Here's how the part is built. I have some questions about the finished solid (model axes, mm). A direction names the side the tool comes from. Round coordinates to 2 decimals unless told otherwise and drop trailing zeros. Loops run counter-clockwise (first coordinate to the right, second up) from the corner with the lowest first, then second, coordinate; pieces in that order, holes last. Notation, with made-up numbers: (62.25, 81) - (71.25, 81) arc R15 ccw to (71.25, 90) - close; hole circle Ø2 at (23.5, -9.75). An arc over 180 degrees is marked (long way). Answer as a JSON object with one key per item and string values. Group by question number.
1) I want a section at A-A, the plane z = 0. Please give me the cut outline in (x, y).
2) Will this pin go through, and if not, where does the flat tip stop? P1, Ø3, axis at x = 7, z = -2.5, coming from the -Y side.
3) If I drill on line 1 along X through (y, z) = (-3.75, -5.5); line 2 along Y through (x, z) = (13.5, 0.25); line 3 along Z through (x, y) = (1, 0.25), over which ranges is the centre line in solid material (lowest first)? Write a range as [from, to].
4) If we mould it in two halves opening along X, with no side actions, what happens to faces 1 (the face through (0, 0, 0)), 2 (the face through (24.74, 6.21, 3.23)), 3 (the face through (21.058, 3.955, -5.158)), 4 (the face through (28, 0, 0))? For each: pulls with the +X half, pulls with the -X half, needs draft (parallel to the pull), parting line crosses it, or undercut.
5) I want a section at C-C, the plane x = 14. Please give me the cut outline in (y, z).
6) Which directions (+Z, -Z, +X, -X, +Y, -Y) give clear straight access to the entire face, cutting with the end or side of a thin tool? Please do faces 5 (the face through (10, -5, 2)), 6 (the face through (15.32, 6.21, 3.23)).
from build123d import *

# Parameters (mm, degrees)
CHAMFER1_SIZE = 0.2
CHAMFER2_SIZE = 0.2
SKETCH4_W     = 1.1
SKETCH4_H     = 2.393770958


with BuildPart() as part:
    # Sketch1 → Revolve1 (revolve)
    with BuildSketch(Plane.XY, mode=Mode.PRIVATE) as revolve1_sk:
        Polygon((0, 0), (0, 5), (10, 5), (10, 7), (28, 7), (28, 0), align=None)
    revolve(revolve1_sk.sketch.rotate(Axis((0, 0, 0), (1, 0, 0)), 90), axis=Axis((0, 0, 0), (1, 0, 0)))

    # Chamfer1
    chamfer1_edges = [part.edges().sort_by_distance(p)[0] for p in [
        (0, 0, -5),
    ]]
    chamfer(chamfer1_edges, length=CHAMFER1_SIZE)

    # Chamfer2
    chamfer2_edges = [part.edges().sort_by_distance(p)[0] for p in [
        (28, 0, -7),
    ]]
    chamfer(chamfer2_edges, length=CHAMFER2_SIZE)

    # Sketch4 → Cut-Revolve1 (revolve, cut)
    with BuildSketch(Plane(origin=(0, 0, 0), x_dir=(1, 0, 0), z_dir=(0, 1, 0)), mode=Mode.PRIVATE) as cut_revolve1_sk:
        with Locations((21.05, 7.696885479)):
            Rectangle(SKETCH4_W, SKETCH4_H)
    revolve(cut_revolve1_sk.sketch.rotate(Axis((0, 0, 0), (1, 0, 0)), 180), axis=Axis((0, 0, 0), (1, 0, 0)), mode=Mode.SUBTRACT)


solid = part.part
Outcome:
{
 "1": {"outline": "(0, -4.8) - (0.2, -5) - (10, -5) - (10, -7) - (20.5, -7) - (20.5, -6.5) - (21.6, -6.5) - (21.6, -7) - (27.8, -7) - (28, -6.8) - (28, 6.8) - (27.8, 7) - (21.6, 7) - (21.6, 6.5) - (20.5, 6.5) - (20.5, 7) - (10, 7) - (10, 5) - (0.2, 5) - (0, 4.8) - close"},
 "2": {"P1": "y = -4.9"},
 "3": {"line 1": "[10, 20.5], [21.6, 28]", "line 2": "[-7, 7]", "line 3": "[-4.99, 4.99]"},
 "4": {"face 1": "pulls with the -X half", "face 2": "needs draft", "face 3": "undercut", "face 4": "pulls with the +X half"},
 "5": {"outline": "circle Ø14 at (0, 0)"},
 "6": {"face 5": "-X", "face 6": "+X, -X"}
}
